Check sheet for the modelled part. Datum: model origin and axes. Units: mm. Round coordinates to 2 decimals unless told otherwise and drop trailing zeros. Loops run counter-clockwise (first coordinate to the right, second up) from the corner with the lowest first, then second, coordinate; pieces in that order, holes last. Notation, with made-up numbers: (40, -21.5) - (44, -21.5) arc R29 cw to (44, 17.5) - close; hole circle Ø4 at (40.25, 40). An arc over 180 degrees is marked (long way). Answer in a Markdown table with one row per item. Add a question column.
(1) Cross-section at A-A on y = 0. Enter the section's corners in (x, z).
(2) Cross-section at C-C on z = -40.5. Enter the section's corners in (x, y), then the cut area to 3 significant figures.
(3) Cross-section at B-B on z = 71. Enter the section's corners in (x, y), then the cut area to 3 significant figures.
(4) Thickness scan on line 1 along X through (y, z) = (-0.5, -39.5); line 2 along Y through (x, z) = (0, 64); line 3 along Y through (x, z) = (82, 127). Record the ranges inside material, lowest first.
(5) Gauge pin test, flat ends, axial feed: pin 1 (3 mm diameter, centred on x = 9.5, y = -6.5, fed in from -Z); pin 2 (12 mm diameter, centred on x = 71.5, y = 3.5, fed in from +Z); pin 3 (4 mm diameter, centred on x = 43, y = 4, fed in from -Z). Record the tip position at first contact, or that the pin passes through.
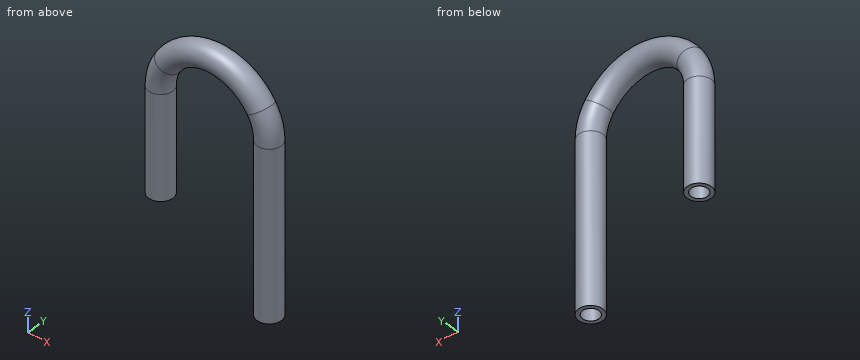
from build123d import *

# Parameters (mm, degrees)
SKETCH1_R   = 11
SKETCH1_R_2 = 7.5


with BuildPart() as part:
    # Sweep1: sweep along a path in Sketch2
    with BuildLine(Plane(origin=(0, 0, 0), x_dir=(1, 0, 0), z_dir=(0, 1, 0))) as sweep1_path:
        Line((0, 0), (0, -93.298854008))
        ThreePointArc((0, -93.298854008), (1.899755617, -106.235968606), (7.438619295, -118.080756266))
        ThreePointArc((7.438619295, -118.080756266), (50, -140.990195136), (92.561380705, -118.080756266))
        ThreePointArc((92.561380705, -118.080756266), (98.100244383, -106.235968606), (100, -93.298854008))
        Line((100, -93.298854008), (100, 59.000000002))
    # Sketch1 → Sweep1 (sweep)
    with BuildSketch(Plane.XY):
        Circle(SKETCH1_R)
        Circle(SKETCH1_R_2, mode=Mode.SUBTRACT)
    sweep(path=sweep1_path.line)


solid = part.part
Answers:
| question | item | result |
|---|---|---|
| 1 | outline | (-11, 0) - (-7.5, 0) - (-7.5, 93.3) arc R52.5 cw to (1.18, 122.21) arc R58.49 cw to (98.82, 122.21) arc R52.5 cw to (107.5, 93.3) - (107.5, -59) - (111, -59) - (111, 93.3) arc R56 ccw to (101.74, 124.14) arc R61.99 ccw to (-1.74, 124.14) arc R56 ccw to (-11, 93.3) - close; (7.5, 0) - (11, 0) - (11, 93.3) arc R34 cw to (16.62, 112.02) arc R39.99 cw to (83.38, 112.02) arc R34 cw to (89, 93.3) - (89, -59) - (92.5, -59) - (92.5, 93.3) arc R37.5 ccw to (86.3, 113.95) arc R43.49 ccw to (13.7, 113.95) arc R37.5 ccw to (7.5, 93.3) - close |
| 2 | outline | circle Ø22 at (100, 0); hole circle Ø15 at (100, 0) |
| 2 | area | 203 mm^2 |
| 3 | outline | circle Ø22 at (0, 0); circle Ø22 at (100, 0); hole circle Ø15 at (0, 0); hole circle Ø15 at (100, 0) |
| 3 | area | 407 mm^2 |
| 4 | line 1 | x = 89.01 to 92.52, 107.48 to 110.99 |
| 4 | line 2 | y = -11 to -7.5, 7.5 to 11 |
| 4 | line 3 | y = -10.8 to -7.21, 7.21 to 10.8 |
| 5 | pin 1 | stops at z = 0 |
| 5 | pin 2 | stops at z = 149.83 |
| 5 | pin 3 | stops at z = 129.41 |
